Could you check a few things on this model? Use its own coordinates, in mm. A direction names the side the tool comes from. Give positions to 0.01 mm unless a question says otherwise; leave off trailing zeros. Loops run counter-clockwise (first coordinate to the right, second up) from the corner with the lowest first, then second, coordinate; pieces in that order, holes last. Notation, with made-up numbers: M 32.25,20.5 L 83.25,20.5 A18 ccw 83.25,26.5 Z; hole C -1.75,-18.75 d9. An arc over 180 degrees is marked long. Answer in a Markdown table with one row per item. Add a question column.
1. If we section it at B-B on x = 45.5: List the corners of the cut face in (y, z) for me, then the cut area to 3 significant figures.
2. If we section it at D-D on x = 80.5: List the corners of the cut face in (y, z) for me, then the cut area to 3 significant figures.
3. If we section it at A-A on y = 0: List the corners of the cut face in (x, z) for me, then the cut area to 3 significant figures.
4. Which directions (+Z, -Z, +X, -X, +Y, -Y) give clear straight access to the entire face, cutting with the end or side of a thin tool? Please do faces 4 (the flat face through (-52, 2, 0)), 5 (the flat face through (61.23, 85.557, 29.635)), 6 (the flat face through (-85.22, -60.99, 29.64)), 7 (the cylindrical face through (-63.49, 63.79, 29.64)).
5. I'm going to push flat-ended pins straight in: pin 1 Ø3 at (y, z) = (79, 8) entering from -X; pin 2 Ø4 at (y, z) = (95.5, 49) entering from -X; pin 3 Ø5 at (y, z) = (47.5, 24.5) entering from -X. Where does each tip first touch, or does it pass through?
6. I need wall thicknesses on line 1 along Z through (x, y) = (41.5, -1.5); line 2 along Y through (x, z) = (0, 1.6); line 3 along Y through (x, z) = (-96.5, 15). Which ranges of each line are inside material? Lowest first, please. Write a range as from..to.
7. If we section it at C-C on y = 31: List the corners of the cut face in (x, z) for me, then the cut area to 3 significant figures.
8. Thinking about a two-plate mould opening in Y: for faces 1 (the flat face through (103.38, -17.133, 29.635)), 2 (the flat face through (60.99, -85.22, 29.64)), 3 (the flat face through (52, 2, 59.97)), which applies, released by +Y, released by -Y, zero draft, split by the parting line, or undercut?
```python
from build123d import *

# Parameters (mm, degrees)
SKETCH1_R           = 150
SKETCH1_R_2         = 120
BOSS_EXTRUDE1_DEPTH = 59.97
BOSS_EXTRUDE2_START = -59.97
SKETCH2_R           = 120
SKETCH2_R_2         = 90
BOSS_EXTRUDE2_DEPTH = 59.97
CUT_EXTRUDE1_START  = -59.97
CUT_EXTRUDE1_DEPTH  = 59.97
CIRPATTERN1_COUNT   = 8
CUT_EXTRUDE2_START  = -49.97
CUT_EXTRUDE2_DEPTH  = 49.97
CIRPATTERN2_COUNT   = 8
BOSS_EXTRUDE3_START = -5
SKETCH6_R           = 90
SKETCH6_R_2         = 40.03
BOSS_EXTRUDE3_DEPTH = 5
SKETCH7_R           = 90
SKETCH7_R_2         = 40.03
BOSS_EXTRUDE4_DEPTH = 5
SKETCH8_R           = 150
SKETCH8_R_2         = 120
CUT_EXTRUDE3_DEPTH  = 80
SKETCH10_W          = 5
SKETCH10_H          = 5
CUT_REVOLVE1_ANGLE  = 30


with BuildPart() as part:
    # Sketch1 → Boss-Extrude1 (new body)
    with BuildSketch(Plane.XY):
        Circle(SKETCH1_R)
        Circle(SKETCH1_R_2, mode=Mode.SUBTRACT)
    extrude(amount=BOSS_EXTRUDE1_DEPTH)

    # Sketch2 → Boss-Extrude2 (add)
    with BuildSketch(Plane.XY.offset(59.97).offset(BOSS_EXTRUDE2_START)):
        Circle(SKETCH2_R)
        Circle(SKETCH2_R_2, mode=Mode.SUBTRACT)
    extrude(amount=BOSS_EXTRUDE2_DEPTH)

    # Sketch3 → Cut-Extrude1 (cut)
    with BuildSketch(Plane.XY.offset(59.97).offset(CUT_EXTRUDE1_START)):
        with BuildLine():
            Line((-15.663143066, 118.973383365), (-19.578928833, 148.716729206))
            ThreePointArc((-19.578928833, 148.716729206), (0, 150), (19.578928833, 148.716729206))
            Line((19.578928833, 148.716729206), (15.663143066, 118.973383365))
            ThreePointArc((15.663143066, 118.973383365), (0, 120), (-15.663143066, 118.973383365))
        make_face()
    cut_extrude1 = extrude(amount=CUT_EXTRUDE1_DEPTH, mode=Mode.SUBTRACT)

    # CirPattern1: Cut-Extrude1 ×8 about axis
    cirpattern1_axis = Axis((0, 0, 0), (0, 0, 1))
    for i in range(1, CIRPATTERN1_COUNT):
        add(cut_extrude1.rotate(cirpattern1_axis, i * 360 / CIRPATTERN1_COUNT), mode=Mode.SUBTRACT)

    # Sketch5 → Cut-Extrude2 (cut)
    with BuildSketch(Plane.XY.offset(54.97).offset(CUT_EXTRUDE2_START)):
        with BuildLine():
            Line((14.714615406, 88.788963804), (24.524359011, 147.98160634))
            ThreePointArc((24.524359011, 147.98160634), (57.402514855, 138.581929877), (87.297456773, 121.980137895))
            Line((87.297456773, 121.980137895), (52.378474064, 73.188082737))
            ThreePointArc((52.378474064, 73.188082737), (34.441508913, 83.149157926), (14.714615406, 88.788963804))
        make_face()
    cut_extrude2 = extrude(amount=CUT_EXTRUDE2_DEPTH, mode=Mode.SUBTRACT)

    # CirPattern2: Cut-Extrude2 ×8 about axis
    cirpattern2_axis = Axis((0, 0, 0), (0, 0, 1))
    for i in range(1, CIRPATTERN2_COUNT):
        add(cut_extrude2.rotate(cirpattern2_axis, i * 360 / CIRPATTERN2_COUNT), mode=Mode.SUBTRACT)

    # Sketch6 → Boss-Extrude3 (add)
    with BuildSketch(Plane.XY.offset(59.97).offset(BOSS_EXTRUDE3_START)):
        Circle(SKETCH6_R)
        Circle(SKETCH6_R_2, mode=Mode.SUBTRACT)
    extrude(amount=BOSS_EXTRUDE3_DEPTH)

    # Sketch7 → Boss-Extrude4 (add)
    with BuildSketch(Plane(origin=(0, 0, 0), x_dir=(-1, 0, 0), z_dir=(0, 0, -1))):
        Circle(SKETCH7_R)
        with Locations(Location((0, 0, 0), (0, 0, 180))):
            Circle(SKETCH7_R_2, mode=Mode.SUBTRACT)
    extrude(amount=-BOSS_EXTRUDE4_DEPTH)

    # Sketch8 → Cut-Extrude3 (cut)
    with BuildSketch(Plane(origin=(0, 0, 0), x_dir=(-1, 0, 0), z_dir=(0, 0, -1))):
        Circle(SKETCH8_R)
        with Locations(Location((0, 0, 0), (0, 0, 180))):
            Circle(SKETCH8_R_2, mode=Mode.SUBTRACT)
    extrude(amount=-CUT_EXTRUDE3_DEPTH, mode=Mode.SUBTRACT)

    # Sketch10 → Cut-Revolve1 (revolve, cut)
    with BuildSketch(Plane(origin=(0, 0, 0), x_dir=(0, 0, -1), z_dir=(0.9865440422698816, -0.16349572673865878, 0))):
        with Locations((-29.985, 117.5)):
            Rectangle(SKETCH10_W, SKETCH10_H)
    revolve(axis=Axis((0, 0, 0), (0, 0, 1)), revolution_arc=CUT_REVOLVE1_ANGLE, mode=Mode.SUBTRACT)


solid = part.part
```
Results:
| question | item | result |
|---|---|---|
| 1 | outline | M -111.04,0 L 111.04,0 L 111.04,5 L -111.04,5 Z; M -111.04,54.97 L 111.04,54.97 L 111.04,59.97 L -111.04,59.97 Z |
| 1 | area | 2,220 mm2 |
| 2 | outline | M -88.99,0 L 88.99,0 L 88.99,59.97 L -88.99,59.97 Z; hole M -57.61,5 L 57.61,5 L 57.61,54.97 L -57.61,54.97 Z |
| 2 | area | 4,920 mm2 |
| 3 | outline | M -120,0 L -40.03,0 L -40.03,5 L -90,5 L -90,54.97 L -40.03,54.97 L -40.03,59.97 L -120,59.97 Z; M 40.03,0 L 120,0 L 120,59.97 L 40.03,59.97 L 40.03,54.97 L 90,54.97 L 90,5 L 40.03,5 Z |
| 3 | area | 4,600 mm2 |
| 4 | face 4 | -Z, +X, -X, +Y, -Y |
| 4 | face 5 | +Y |
| 4 | face 6 | -X |
| 4 | face 7 | none |
| 5 | pin 1 | x = -91.62 |
| 5 | pin 2 | x = -75.22 |
| 5 | pin 3 | through |
| 6 | line 1 | 0..5, 54.97..59.97 |
| 6 | line 2 | -120..-40.03, 40.03..120 |
| 6 | line 3 | -71.33..-69.06, -15.99..15.99, 69.06..71.33 |
| 7 | outline | M -115.93,0 L -25.33,0 L -25.33,5 L -115.93,5 Z; M -115.93,54.97 L -25.33,54.97 L -25.33,59.97 L -115.93,59.97 Z; M 25.33,0 L 115.93,0 L 115.93,5 L 25.33,5 Z; M 25.33,54.97 L 115.93,54.97 L 115.93,59.97 L 25.33,59.97 Z |
| 7 | area | 1,810 mm2 |
| 8 | face 1 | undercut |
| 8 | face 2 | released by -Y |
| 8 | face 3 | zero draft |
